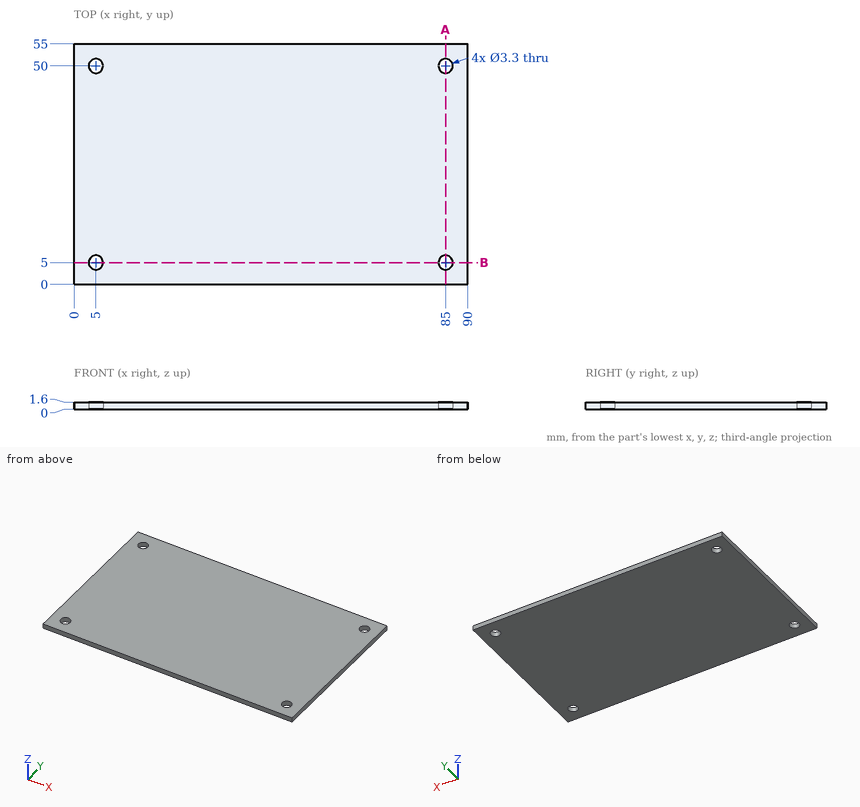
Source: three-view drawing plus pictorial views. Frame: mm from the lowest corner of the part. Give positions to 0.01 mm unless a question says otherwise; leave off trailing zeros. Order: outer loops, then holes, each group sorted by start corner. A loop starts at its lowest first (then second) coordinate and runs counter-clockwise, first axis right, second up. Notation, with made-up numbers: (11.5, -29.5) -> (33.5, -29.5) arc R13 cw to (33.5, -11.5) -> close; hole circle Ø10 at (4, 30). An arc over 180 degrees is marked (long way). Write each question's results on one line, items separated by ' | '. Start each with the question number.
Item 1: Contact query for a flat-ended pin moving along its axis: P1, Ø2.5, axis at x = 85, y = 50, coming from the -Z side. Output: stop coordinate, or through.
Item 2: Line query: line 1 (Y direction, x = 5, z = 0.65); line 2 (X direction, y = 49, z = 1.2); line 3 (X direction, y = 48.5, z = 1.45). Output: solid intervals per line, ascending.
Item 3: Cut plane A-A on x = 85. Return the cut outline in (y, z), then the cut area to 3 significant figures.
Item 4: Cut plane B-B on y = 5. Return the cut outline in (x, z), then the cut area to 3 significant figures.
Established:
1) P1: through
2) line 1: 0 to 3.35, 6.65 to 48.35, 51.65 to 55 | line 2: 0 to 3.69, 6.31 to 83.69, 86.31 to 90 | line 3: 0 to 4.31, 5.69 to 84.31, 85.69 to 90
3) outline: (0, 0) -> (3.35, 0) -> (3.35, 1.6) -> (0, 1.6) -> close; (6.65, 0) -> (48.35, 0) -> (48.35, 1.6) -> (6.65, 1.6) -> close; (51.65, 0) -> (55, 0) -> (55, 1.6) -> (51.65, 1.6) -> close | area: 77.4 mm^2
4) outline: (0, 0) -> (3.35, 0) -> (3.35, 1.6) -> (0, 1.6) -> close; (6.65, 0) -> (83.35, 0) -> (83.35, 1.6) -> (6.65, 1.6) -> close; (86.65, 0) -> (90, 0) -> (90, 1.6) -> (86.65, 1.6) -> close | area: 133 mm^2
